Design review of the part shown in the three views and the two pictorial views. Dimensions are in mm from the part's minimum x, y and z. Coordinates: 2 decimals unless noted, no trailing zeros. Loops run counter-clockwise (first coordinate to the right, second up) from the corner with the lowest first, then second, coordinate; pieces in that order, holes last. Notation, with made-up numbers: (67.25, 31) -> (113.25, 31) arc R8 cw to (113.25, 45) -> close; hole circle Ø1 at (-25.5, 47). An arc over 180 degrees is marked (long way). Answer in a Markdown table with one row per item.
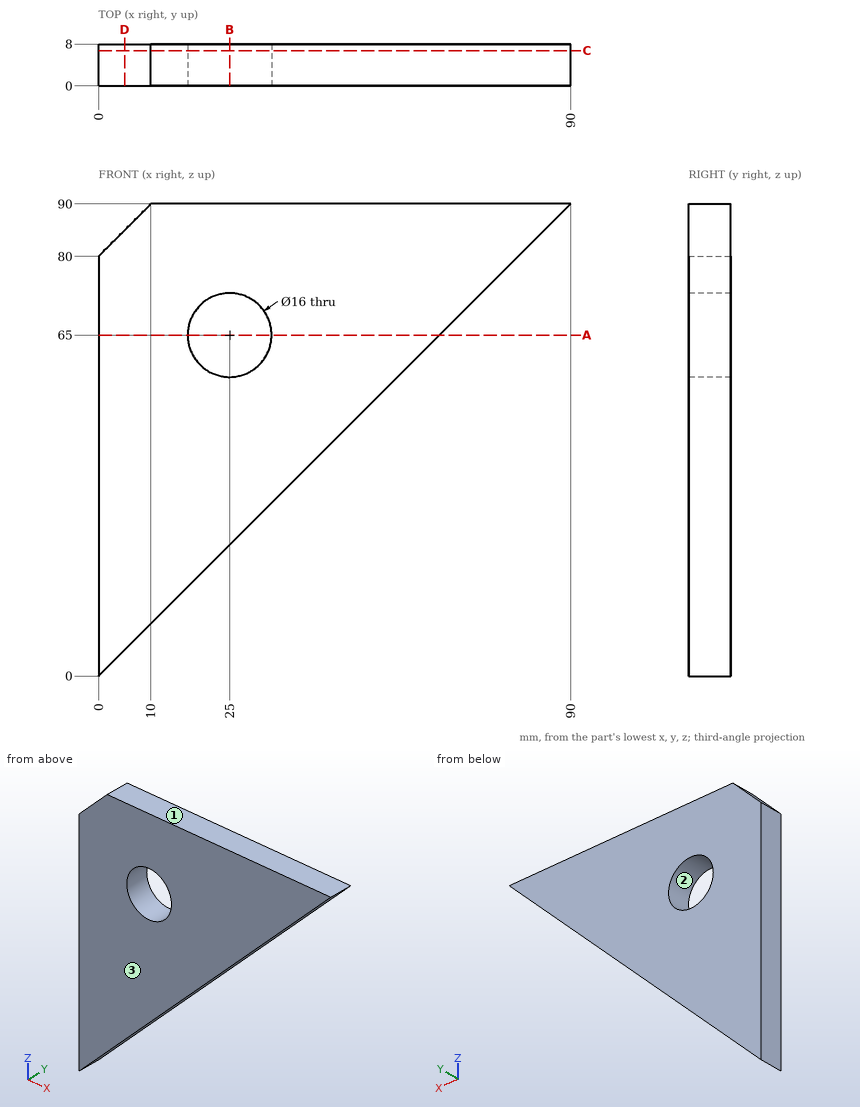
Item 1: Insertion check: pin 1 (2 mm diameter, centred on x = 28.5, y = 6.5, fed in from -Z). The pin has a flat end and moves straight along its axis. Give the tip position at first contact, or say it passes through.
Worked answers:
| item | result |
|---|---|
| pin 1 | z = 27.5 |
Item 2: Take a section at D-D, the plane x = 5. State the section outline as (y, z) points.
Worked answers:
| item | result |
|---|---|
| outline | (0, 5) -> (8, 5) -> (8, 85) -> (0, 85) -> close |
Item 3: Take a section at C-C, the plane y = 6.75. State the section outline as (x, z) points.
Worked answers:
| item | result |
|---|---|
| outline | (0, 0) -> (90, 90) -> (10, 90) -> (0, 80) -> close; hole circle Ø16 at (25, 65) |
Item 4: Take a section at A-A, the plane z = 65. State the section outline as (x, y) points, and give its area (3 significant figures).
Worked answers:
| item | result |
|---|---|
| outline | (0, 0) -> (17, 0) -> (17, 8) -> (0, 8) -> close; (33, 0) -> (65, 0) -> (65, 8) -> (33, 8) -> close |
| area | 392 mm² |
Item 5: For L1, parallel to X at y = 0.5, z = 33; L2, parallel to Z at x = 25, y = 2.5; L3, parallel to X at y = 5.75, z = 65, list the stretches that pass through material, from the lowest coordinate up.
Worked answers:
| item | result |
|---|---|
| L1 | 0 to 33 |
| L2 | 25 to 57, 73 to 90 |
| L3 | 0 to 17, 33 to 65 |
Item 6: The part is to be moulded in two halves that separate along Z. For the marked faces 1, 2 and 3, say which applies: +Z half, -Z half, draft (parallel to the pull), parting line (faces both ways), or undercut.
Worked answers:
| item | result |
|---|---|
| face 1 | +Z half |
| face 2 | undercut |
| face 3 | draft |
Item 7: Take a section at B-B, the plane x = 25. State the section outline as (y, z) points.
Worked answers:
| item | result |
|---|---|
| outline | (0, 25) -> (8, 25) -> (8, 57) -> (0, 57) -> close; (0, 73) -> (8, 73) -> (8, 90) -> (0, 90) -> close |
